Part model, mm, in its own coordinate system. Round coordinates to 2 decimals unless told otherwise and drop trailing zeros. Write each loop counter-clockwise with the first axis right and the second up, starting at its lowest first coordinate (ties: lowest second). Pieces come first, ordered by that corner, then holes. Notation, with made-up numbers: (67, 11) -> (87, 11) arc R22 cw to (87, 21) -> close; hole circle Ø4 at (31, 19.5). An arc over 180 degrees is marked (long way). Return JSON: item names as keys, results as strings. Group by question number.
(1) Mould opens along X. For faces 1 (the cylindrical face through (12.932, -5.362, -0.042)), 2 (the flat face through (0, 33, -3)), 3 (the cylindrical face through (24, -23, 0)) say: +X half, -X half, draft (parallel to the pull), parting line (faces both ways), or undercut.
(2) Drill centre lines: L1, parallel to X at y = -0.5, z = 1.9; L2, parallel to Y at x = 0, z = -0.5; L3, parallel to Y at x = 2, z = -0.15. Where is each one in solid material? Low to high. Write a range as from..to.
(3) Saw through at A-A (x = 0). List the corners of the cut face in (y, z), plus the area to 3 significant figures.
(4) Saw through at B-B (y = 0). List the corners of the cut face in (x, z).
(5) Saw through at C-C (z = -1.6). List the corners of the cut face in (x, y).
from build123d import *

# Parameters (mm, degrees)
SKETCH1_R           = 14
BOSS_EXTRUDE1_DEPTH = 3


with BuildPart() as part:
    # Sketch1 → Boss-Extrude1 (new, symmetric)
    with BuildSketch(Plane.XY):
        with BuildLine():
            Line((-25, 90), (25, 90))
            Line((25, 90), (25, -20))
            ThreePointArc((25, -20), (23.535533906, -23.535533906), (20, -25))
            Line((20, -25), (-20, -25))
            ThreePointArc((-20, -25), (-23.535533906, -23.535533906), (-25, -20))
            Line((-25, -20), (-25, 90))
        make_face()
        Circle(SKETCH1_R, mode=Mode.SUBTRACT)
    extrude(amount=BOSS_EXTRUDE1_DEPTH, both=True)


solid = part.part
Computed values:
{
 "1": {"face 1": "undercut", "face 2": "draft", "face 3": "+X half"},
 "2": {"L1": "-25..-13.99, 13.99..25", "L2": "-25..-14, 14..90", "L3": "-25..-13.86, 13.86..90"},
 "3": {"outline": "(-25, -3) -> (-14, -3) -> (-14, 3) -> (-25, 3) -> close; (14, -3) -> (90, -3) -> (90, 3) -> (14, 3) -> close", "area": "522 mm2"},
 "4": {"outline": "(-25, -3) -> (-14, -3) -> (-14, 3) -> (-25, 3) -> close; (14, -3) -> (25, -3) -> (25, 3) -> (14, 3) -> close"},
 "5": {"outline": "(-25, -20) arc R5 ccw to (-20, -25) -> (20, -25) arc R5 ccw to (25, -20) -> (25, 90) -> (-25, 90) -> close; hole circle Ø28 at (0, 0)"}
}
